Check sheet for the modelled part. Datum: model origin and axes. Units: mm. Face numbers are marked on the shaded views. Round coordinates to 2 decimals unless told otherwise and drop trailing zeros. Write each loop counter-clockwise with the first axis right and the second up, starting at its lowest first coordinate (ties: lowest second). Pieces come first, ordered by that corner, then holes. Notation, with made-up numbers: M -21,64 L 18,64 A16 ccw 18,92 Z; hole C -5.75,2 d6. An arc over 180 degrees is marked long. Put each result on its own line as item: value.
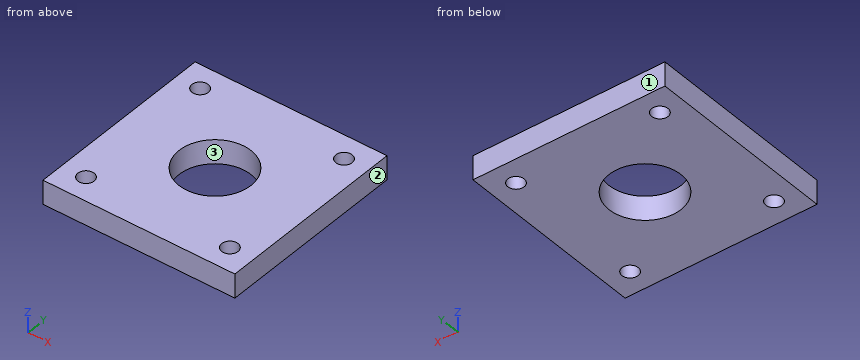
```python
from build123d import *

# Parameters (mm, degrees)
SKETCH1_W             = 80
SKETCH1_H             = 80
BOSS_EXTRUDE1_DEPTH   = 10
M8_TAPPED_HOLE1_D     = 6.8
M8_TAPPED_HOLE1_DEPTH = 19.75
M8_TAPPED_HOLE1_TIP   = 2.042926105
SKETCH5_R             = 15
CUT_EXTRUDE1_DEPTH    = 10


with BuildPart() as part:
    # Sketch1 → Boss-Extrude1 (new body)
    with BuildSketch(Plane.XY):
        Rectangle(SKETCH1_W, SKETCH1_H)
    extrude(amount=BOSS_EXTRUDE1_DEPTH)

    # M8 Tapped Hole1
    with Locations(Plane.XY.offset(10)):
        with Locations((-30, 30), (30, 30), (30, -30), (-30, -30)):
            Hole(M8_TAPPED_HOLE1_D / 2, depth=M8_TAPPED_HOLE1_DEPTH)
            with Locations((0, 0, -(M8_TAPPED_HOLE1_DEPTH + M8_TAPPED_HOLE1_TIP / 2))):  # 118° drill point
                Cone(0, M8_TAPPED_HOLE1_D / 2, M8_TAPPED_HOLE1_TIP, mode=Mode.SUBTRACT)

    # Sketch5 → Cut-Extrude1 (cut)
    with BuildSketch(Plane.XY.offset(10)):
        Circle(SKETCH5_R)
    extrude(amount=-CUT_EXTRUDE1_DEPTH, mode=Mode.SUBTRACT)


solid = part.part
```
1. Cross-section at A-A (x = 0). Enter the section's corners in (y, z), then the cut area to 3 significant figures.
Computed values:
outline: M -40,0 L -15,0 L -15,10 L -40,10 Z; M 15,0 L 40,0 L 40,10 L 15,10 Z
area: 500 mm2
2. Cross-section at C-C (z = 3.25). Enter the section's corners in (x, y), then the cut area to 3 significant figures.
Computed values:
outline: M -40,-40 L 40,-40 L 40,40 L -40,40 Z; hole C -30,-30 d6.8; hole C -30,30 d6.8; hole C 0,0 d30; hole C 30,-30 d6.8; hole C 30,30 d6.8
area: 5,550 mm2
3. Depth check by flat-ended pin: pin 1 Ø11 at (x, y) = (-30, -30) entering from -Z. Enter the tip coordinate at first touch or a pass-through.
Computed values:
pin 1: stops at z = 0
4. Release check for a two-part mould opening along X. For the marked faces 1, 2 and 3 record: +X half, -X half, draft (parallel to the pull), parting line (faces both ways), or undercut.
Computed values:
face 1: draft
face 2: +X half
face 3: undercut
5. Cross-section at B-B (y = -30). Enter the section's corners in (x, z).
Computed values:
outline: M -40,0 L -33.4,0 L -33.4,10 L -40,10 Z; M -26.6,0 L 26.6,0 L 26.6,10 L -26.6,10 Z; M 33.4,0 L 40,0 L 40,10 L 33.4,10 Z
6. Scan lines: probe 1 along Y at (x, z) = (30, 4.75); probe 2 along Y at (x, z) = (28.5, 9); probe 3 along Y at (x, z) = (0, 7.75). Record each from-to range of solid material in increasing order.
Computed values:
probe 1: y = -40 to -33.4, -26.6 to 26.6, 33.4 to 40
probe 2: y = -40 to -33.05, -26.95 to 26.95, 33.05 to 40
probe 3: y = -40 to -15, 15 to 40
